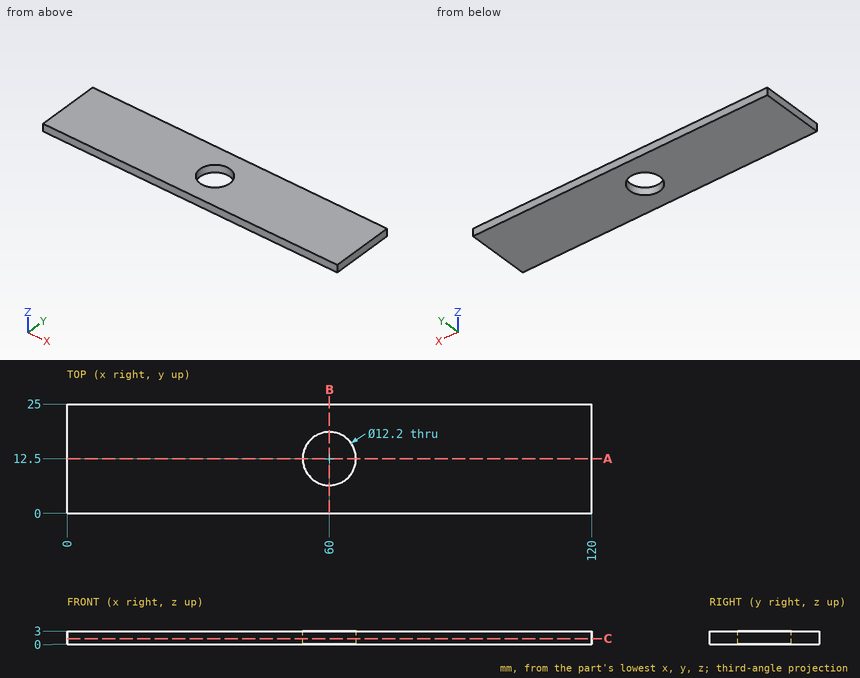
Source: three-view drawing plus pictorial views. Frame: mm from the lowest corner of the part. Round coordinates to 2 decimals unless told otherwise and drop trailing zeros. Order: outer loops, then holes, each group sorted by start corner. A loop starts at its lowest first (then second) coordinate and runs counter-clockwise, first axis right, second up. Notation, with made-up numbers: M 81.25,-32.5 L 93.25,-32.5 A25 ccw 93.25,-19.5 Z; hole C 4.5,-11.75 d7. An arc over 180 degrees is marked long. One line per item, written item: value.
(1) Cut plane A-A (y = 12.5). Return the cut outline in (x, z).
Result sheet:
outline: M 0,0 L 53.9,0 L 53.9,3 L 0,3 Z; M 66.1,0 L 120,0 L 120,3 L 66.1,3 Z
(2) Cut plane B-B (x = 60). Return the cut outline in (y, z).
Result sheet:
outline: M 0,0 L 6.4,0 L 6.4,3 L 0,3 Z; M 18.6,0 L 25,0 L 25,3 L 18.6,3 Z
(3) Pin query (flat end, axial travel): P1, Ø10, axis at x = 60, y = 12.5, coming from the +Z side. Return the tip coordinate at first contact, or that it passes through.
Result sheet:
P1: through
(4) Line query: probe 1 along Y at (x, z) = (60, 2.4); probe 2 along X at (y, z) = (12.25, 1.6); probe 3 along X at (y, z) = (10.75, 0.85). Output: solid intervals per line, ascending. Write a range as [from, to].
Result sheet:
probe 1: [0, 6.4], [18.6, 25]
probe 2: [0, 53.91], [66.09, 120]
probe 3: [0, 54.16], [65.84, 120]
(5) Cut plane C-C (z = 1.3). Return the cut outline in (x, y).
Result sheet:
outline: M 0,0 L 120,0 L 120,25 L 0,25 Z; hole C 60,12.5 d12.2
